Can you work these out from the model? Positions are in its coordinate system, mm. Give positions to 0.01 mm unless a question says otherwise; leave off trailing zeros. Order: outer loops, then holes, each group sorted by start corner. A loop starts at its lowest first (then second) coordinate and runs counter-clockwise, first axis right, second up. Notation, with made-up numbers: (-2, 52.5) - (14, 52.5) arc R7 cw to (14, 57.5) - close; hole circle Ø5 at (40.5, 54). An arc over 180 degrees is marked (long way). Answer as CSV lines item,"result".
```python
from build123d import *

# Parameters (mm, degrees)
SKETCH1_W                      = 150
SKETCH1_H                      = 820
BOSS_EXTRUDE1_DEPTH            = 30
M24_THREADED_HOLE1_D           = 21
M24_THREADED_HOLE1_ON_FACE_2_D = 21


with BuildPart() as part:
    # Sketch1 → Boss-Extrude1 (new body)
    with BuildSketch(Plane.XY):
        with Locations((75, 410)):
            Rectangle(SKETCH1_W, SKETCH1_H)
    extrude(amount=BOSS_EXTRUDE1_DEPTH)

    # M24 Threaded hole1 (through all)
    with Locations(Plane(origin=(75, 780, 30), x_dir=(1, 0, 0), z_dir=(0, 0, 1))):
        with Locations((0, 0), (0, -740)):
            Hole(M24_THREADED_HOLE1_D / 2)

    # M24 Threaded hole1 on face 2 (through all)
    with Locations(Plane(origin=(283.451995804, 183.295208972, 0), x_dir=(1, 0, 0), z_dir=(0, 0, 1))):
        with Locations((0, 0)):
            Hole(M24_THREADED_HOLE1_ON_FACE_2_D / 2)


solid = part.part
```
1) I want a section at A-A on x = 75. Write out the boundary of the cut face in (y, z).
Answer block:
outline,"(0, 0) - (29.5, 0) - (29.5, 30) - (0, 30) - close; (50.5, 0) - (769.5, 0) - (769.5, 30) - (50.5, 30) - close; (790.5, 0) - (820, 0) - (820, 30) - (790.5, 30) - close"
2) If we mould it in two halves opening along X, with no side actions, what happens to faces 1 (the flat face through (150, 404, 15)), 2 (the flat face through (0, 404, 15)), 3 (the flat face through (74, 0, 15)), 4 (the cylindrical face through (83.33, 773.61, 14.79))? For each: +X half, -X half, draft (parallel to the pull), parting line (faces both ways), or undercut.
Answer block:
face 1,"+X half"
face 2,"-X half"
face 3,"draft"
face 4,"undercut"
3) I want a section at B-B on y = 780. Write out the boundary of the cut face in (x, z), plus the area to 3 significant figures.
Answer block:
outline,"(0, 0) - (64.5, 0) - (64.5, 30) - (0, 30) - close; (85.5, 0) - (150, 0) - (150, 30) - (85.5, 30) - close"
area,"3,870 mm2"
4) I need wall thicknesses on line 1 along Y through (x, z) = (75, 22); line 2 along X through (y, z) = (780, 8); line 3 along Y through (x, z) = (65.5, 23.75). Which ranges of each line are inside material? Lowest first, please. Write a range as [from, to].
Answer block:
line 1,"[0, 29.5], [50.5, 769.5], [790.5, 820]"
line 2,"[0, 64.5], [85.5, 150]"
line 3,"[0, 35.53], [44.47, 775.53], [784.47, 820]"
